The figure shows three views and two pictorial views of one solid part (mm, origin at its lowest corner). Answer the questions. A direction names the side the tool comes from. Coordinates: 2 decimals unless noted, no trailing zeros. Order: outer loops, then holes, each group sorted by start corner. A loop starts at its lowest first (then second) coordinate and runs counter-clockwise, first axis right, second up. Notation, with made-up numbers: (82.25, 49) -> (87.25, 49) arc R19 cw to (87.25, 63) -> close; hole circle Ø4 at (85.5, -40). An arc over 180 degrees is marked (long way). Return JSON: item names as keys, results as strings.
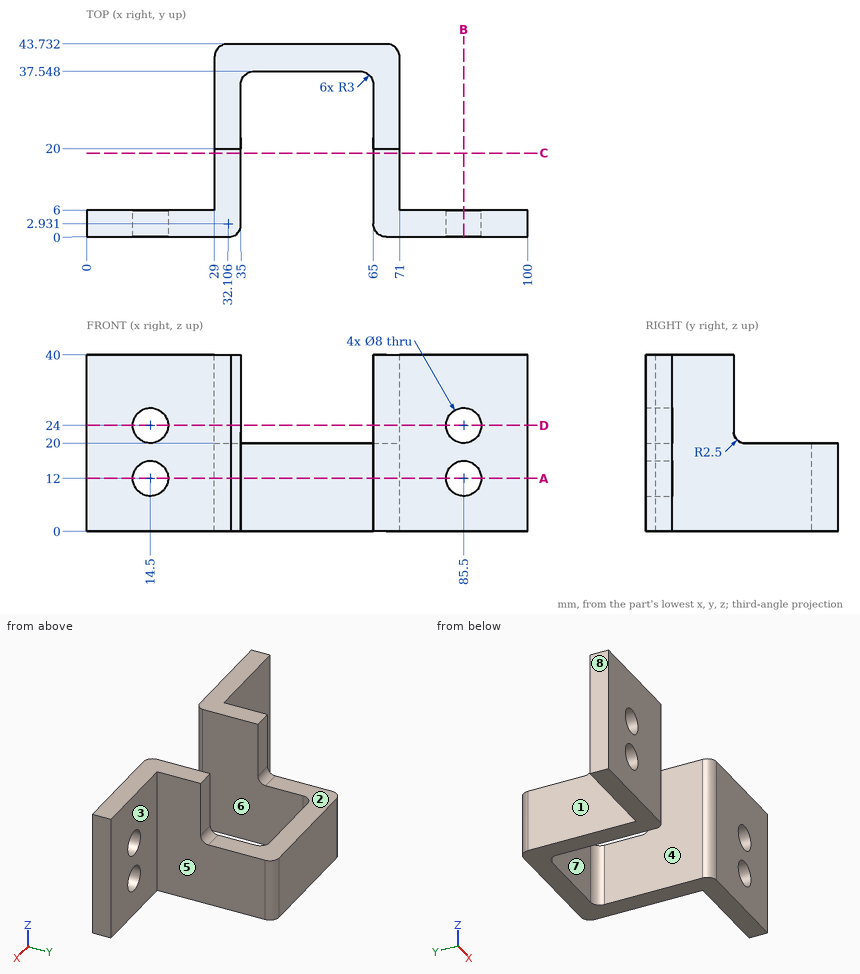
Item 1: Which of the six approach directions +Z, -Z, +X, -X, +Y, -Y give full straight-line access (tool end or side, diameter ignored) to the marked faces 1, 2, 3 and 4?
Answer list:
{"face 1": "+Z, -Z, -X, +Y", "face 2": "+Z, +X, -X, +Y", "face 3": "+Z, -Z, +X, +Y", "face 4": "+Z, -Z, -Y"}
Item 2: Find the intervals of material crossed by probe 1 along Z at (x, y) = (14.5, 4.2); probe 2 along X at (y, z) = (14, 19.5); probe 3 along Z at (x, y) = (30, 41), in increasing order.
Answer list:
{"probe 1": "0 to 8, 16 to 20, 28 to 40", "probe 2": "29 to 35, 65 to 71", "probe 3": "0 to 20"}
Item 3: Flat-ended cylindrical pins translate along their axes: pin 1 (1 mm diameter, centred on x = 44, y = 35.5, fed in from -Z); pin 2 (9 mm diameter, centred on x = 14.5, z = 24, fed in from +Y); pin 3 (6.5 mm diameter, centred on x = 32, z = 28, fed in from +Y); pin 4 (17.5 mm diameter, centred on y = 22, z = 23, fed in from -X). Find the tip coordinate at first contact, or state that the pin passes through.
Answer list:
{"pin 1": "through", "pin 2": "y = 6", "pin 3": "y = 20", "pin 4": "x = 29"}
Item 4: The part is cut by section A-A on z = 12. Determine the outline of the cut face in (x, y), plus the area to 3 significant figures.
Answer list:
{"outline": "(0, 0) -> (10.5, 0) -> (10.5, 6) -> (0, 6) -> close; (18.5, 0) -> (32.75, 0) arc R3 ccw to (35, 2.14) -> (35, 34.55) arc R3 cw to (38, 37.55) -> (62, 37.55) arc R3 cw to (65, 34.55) -> (65, 3) arc R3 ccw to (68, 0) -> (81.5, 0) -> (81.5, 6) -> (71, 6) -> (71, 40.73) arc R3 ccw to (68, 43.73) -> (32, 43.73) arc R3 ccw to (29, 40.73) -> (29, 6) -> (18.5, 6) -> close; (89.5, 0) -> (100, 0) -> (100, 6) -> (89.5, 6) -> close", "area": "959 mm2"}
Item 5: Determine the mould class of the marked faces 5, 6, 7 and 8 for opening direction X: pulls with the +X half, pulls with the -X half, needs draft (parallel to the pull), parting line crosses it, or undercut.
Answer list:
{"face 5": "pulls with the +X half", "face 6": "undercut", "face 7": "undercut", "face 8": "pulls with the -X half"}
Item 6: The part is cut by section D-D on z = 24. Determine the outline of the cut face in (x, y).
Answer list:
{"outline": "(0, 0) -> (10.5, 0) -> (10.5, 6) -> (0, 6) -> close; (18.5, 0) -> (32.75, 0) arc R3 ccw to (35, 2.14) -> (35, 20) -> (29, 20) -> (29, 6) -> (18.5, 6) -> close; (65, 3) arc R3 ccw to (68, 0) -> (81.5, 0) -> (81.5, 6) -> (71, 6) -> (71, 20) -> (65, 20) -> close; (89.5, 0) -> (100, 0) -> (100, 6) -> (89.5, 6) -> close"}
Item 7: The part is cut by section B-B on x = 85.5. Determine the outline of the cut face in (y, z), plus the area to 3 significant figures.
Answer list:
{"outline": "(0, 0) -> (6, 0) -> (6, 8) -> (0, 8) -> close; (0, 16) -> (6, 16) -> (6, 20) -> (0, 20) -> close; (0, 28) -> (6, 28) -> (6, 40) -> (0, 40) -> close", "area": "144 mm2"}
Item 8: The part is cut by section C-C on y = 19. Determine the outline of the cut face in (x, z).
Answer list:
{"outline": "(29, 0) -> (35, 0) -> (35, 40) -> (29, 40) -> close; (65, 0) -> (71, 0) -> (71, 40) -> (65, 40) -> close"}
